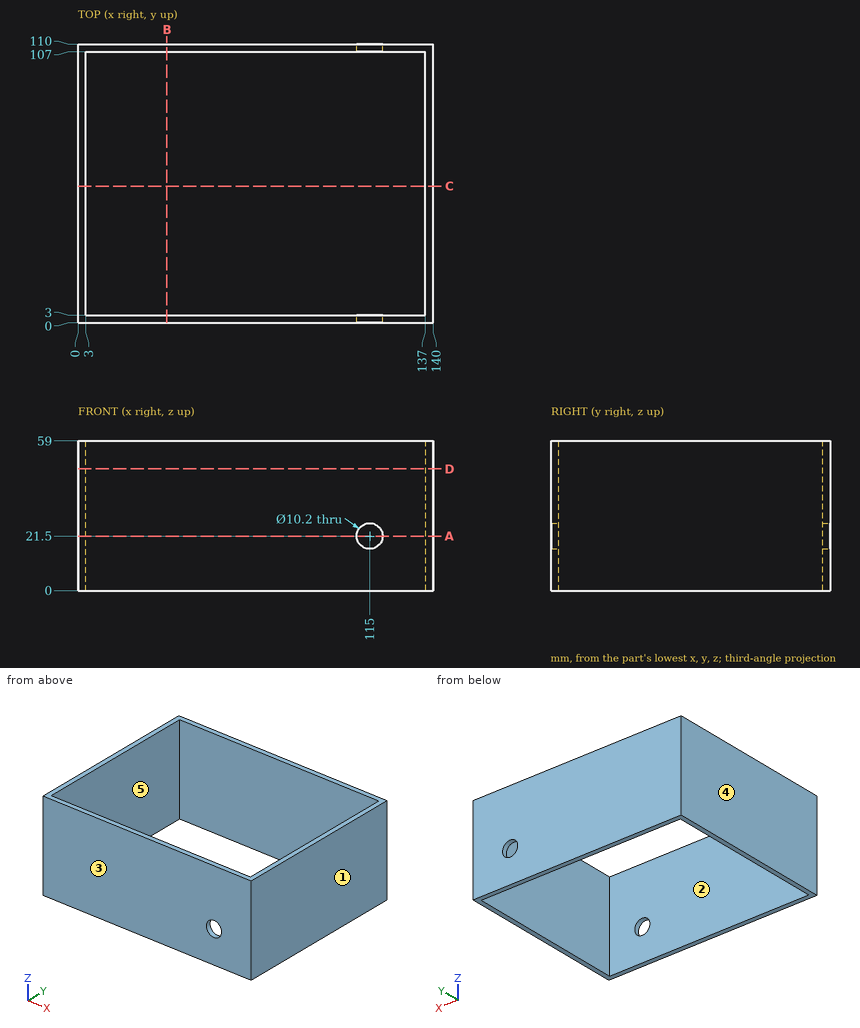
Job drawing, mm, ordinate dimensions from the low corner. One solid piece. A direction names the side the tool comes from. Round coordinates to 2 decimals unless told otherwise and drop trailing zeros. Order: outer loops, then holes, each group sorted by start corner. A loop starts at its lowest first (then second) coordinate and runs counter-clockwise, first axis right, second up. Notation, with made-up numbers: (21, -40) - (68, -40) arc R24 ccw to (68, -13) - close; hole circle Ø5 at (78.5, 10). An arc over 180 degrees is marked (long way). Use CSV: the item, a comma, the result in double quotes. Start each with the question number.
1) Saw through at A-A (z = 21.5). List the corners of the cut face in (x, y).
2) Saw through at C-C (y = 54). List the corners of the cut face in (x, z).
3) Saw through at D-D (z = 48). List the corners of the cut face in (x, y).
4) Saw through at B-B (x = 35). List the corners of the cut face in (y, z).
5) Tool access for the marked faces 1 and 2: list every direction of +Z, -Z, +X, -X, +Y, -Y with a clear straight run to the whole face (end or side of a thin tool).
6) Wall check: L1, parallel to X at y = 58.5, z = 27; L2, parallel to Z at x = 115, y = 1.4; L3, parallel to Y at x = 80, z = 56. Give the ranges that are in metal, low to high. Write a range as [from, to].
7) Two-plate mould, pull along X, no slides. Class the marked faces 3, 4 and 5: pulls with the +X half, pulls with the -X half, needs draft (parallel to the pull), parting line crosses it, or undercut.
Values follow:
1,outline,"(0, 0) - (109.9, 0) - (109.9, 3) - (3, 3) - (3, 107) - (109.9, 107) - (109.9, 110) - (0, 110) - close; (120.1, 0) - (140, 0) - (140, 110) - (120.1, 110) - (120.1, 107) - (137, 107) - (137, 3) - (120.1, 3) - close"
2,outline,"(0, 0) - (3, 0) - (3, 59) - (0, 59) - close; (137, 0) - (140, 0) - (140, 59) - (137, 59) - close"
3,outline,"(0, 0) - (140, 0) - (140, 110) - (0, 110) - close; hole (3, 3) - (137, 3) - (137, 107) - (3, 107) - close"
4,outline,"(0, 0) - (3, 0) - (3, 59) - (0, 59) - close; (107, 0) - (110, 0) - (110, 59) - (107, 59) - close"
5,face 1,"+Z, -Z, +X, +Y, -Y"
5,face 2,"+Z, -Z"
6,L1,"x = [0, 3], [137, 140]"
6,L2,"z = [0, 16.4], [26.6, 59]"
6,L3,"y = [0, 3], [107, 110]"
7,face 3,"needs draft"
7,face 4,"pulls with the -X half"
7,face 5,"undercut"
